Geometry: final body of the model. Coordinates: model frame, mm. Face numbers are marked on the shaded views. A direction names the side the tool comes from. Coordinates: 2 decimals unless noted, no trailing zeros. Loops run counter-clockwise (first coordinate to the right, second up) from the corner with the lowest first, then second, coordinate; pieces in that order, holes last. Notation, with made-up numbers: (77, 63) -> (100, 63) arc R11 cw to (100, 71) -> close; hole circle Ø11 at (-26, 2). An arc over 180 degrees is marked (long way). One line per item, written item: value. Start each with the question number.
Item 1: Contact query for flat-ended pins moving along their axis: pin 1 Ø2.5 at (x, y) = (-9, 34) entering from -Z; pin 2 Ø1.3 at (x, y) = (10.5, 7) entering from -Z. Output: stop coordinate, or through.
Item 2: Section query A-A on x = 0. Return loops of the section in (y, z), then the cut area to 3 significant figures.
Item 3: Set-up query: the marked faces 1, 2 and 3. Return all of +Z, -Z, +X, -X, +Y, -Y with unobstructed straight access to the full face (end or side cutting, diameter ignored); none if empty.
Item 4: Mould query, pull axis X, two halves, no side actions, for the marked faces 4, 5, 6 and 7. Classes: +X half, -X half, draft (parallel to the pull), parting line (faces both ways), or undercut.
Item 5: Ray query, probe 1 along Y at (x, z) = (0, 6.4); probe 2 along X at (y, z) = (21, 6.5); probe 3 along Y at (x, z) = (4.75, 4.75). Return the intervals inside material, ascending. Write a range as from..to.
Item 6: Section query B-B on y = 25.5. Return loops of the section in (x, z).
Item 7: Section query C-C on z = 3. Give the number of separate pieces and of enclosed holes in the cut face, then the cut area to 3 significant figures.
from build123d import *

# Parameters (mm, degrees)
EXTRUDE_1_DEPTH      = 7
EXTRUDE_1_DEPTH_BACK = 7
SKETCH_2_R           = 1.55
SKETCH_2_R_2         = 1.3
SKETCH_2_W           = 15.316718428
SKETCH_2_H           = 46.633436854
CUT_EXTRUDE_1_DEPTH  = 60.640590205
SKETCH_4_W           = 3.5
SKETCH_4_H           = 46.633436854
CUT_EXTRUDE_2_DEPTH  = 45.654227139
FILLET_1_R           = 2


with BuildPart() as part:
    # 草图2 → 凸台-拉伸1 (new, two sides: drawn at the far end of the back side and taken through both)
    with BuildSketch(Plane.XY.offset(-EXTRUDE_1_DEPTH_BACK)):
        with BuildLine():
            Line((9, 37), (-9, 37))
            ThreePointArc((-9, 37), (-11.121320344, 36.121320344), (-12, 34))
            Line((-12, 34), (-12, -18))
            ThreePointArc((-12, -18), (-11.121320344, -20.121320344), (-9, -21))
            Line((-9, -21), (9, -21))
            ThreePointArc((9, -21), (11.121320344, -20.121320344), (12, -18))
            Line((12, -18), (12, 34))
            ThreePointArc((12, 34), (11.121320344, 36.121320344), (9, 37))
        make_face()
        with Locations((-9, -18)):
            Circle(SKETCH_2_R, mode=Mode.SUBTRACT)
        with Locations((0, -18)):
            Circle(SKETCH_2_R_2, mode=Mode.SUBTRACT)
        with Locations((9, -18)):
            Circle(SKETCH_2_R, mode=Mode.SUBTRACT)
        with Locations((0, 8)):
            Rectangle(SKETCH_2_W, SKETCH_2_H, mode=Mode.SUBTRACT)
        with Locations((9, 34)):
            Circle(SKETCH_2_R, mode=Mode.SUBTRACT)
        with Locations((-9, 34)):
            Circle(SKETCH_2_R, mode=Mode.SUBTRACT)
    extrude(amount=EXTRUDE_1_DEPTH + EXTRUDE_1_DEPTH_BACK)

    # 草图3 → 切除-拉伸1 (cut, through all)
    with BuildSketch(Plane.XZ.offset(21)):
        with BuildLine():
            Line((-12, 0.5), (-5.979130372, 0.5))
            ThreePointArc((-5.979130372, 0.5), (0, 6), (5.979130372, 0.5))
            Line((5.979130372, 0.5), (12, 0.5))
            Line((12, 0.5), (12, -7))
            Line((12, -7), (-12, -7))
            Line((-12, -7), (-12, 0.5))
        make_face()
    extrude(amount=-CUT_EXTRUDE_1_DEPTH, mode=Mode.SUBTRACT)

    # 草图4 → 切除-拉伸2 (cut, through all)
    with BuildSketch(Plane.ZY.offset(12)):
        with Locations((2.25, 8)):
            Rectangle(SKETCH_4_W, SKETCH_4_H)
    extrude(amount=-CUT_EXTRUDE_2_DEPTH, mode=Mode.SUBTRACT)

    # 圆角1
    fillet_1_edges = [part.edges().sort_by_distance(p)[0] for p in [
        (7.658359214, 31.316718427, 5.5),
        (-7.658359214, 31.316718427, 5.5),
        (7.658359214, -15.316718427, 5.5),
        (-7.658359214, -15.316718427, 5.5),
        (-9.829179607, 31.316718427, 4),
        (-9.829179607, -15.316718427, 4),
        (9.829179607, -15.316718427, 4),
        (9.829179607, 31.316718427, 4),
    ]]
    fillet(fillet_1_edges, radius=FILLET_1_R)


solid = part.part
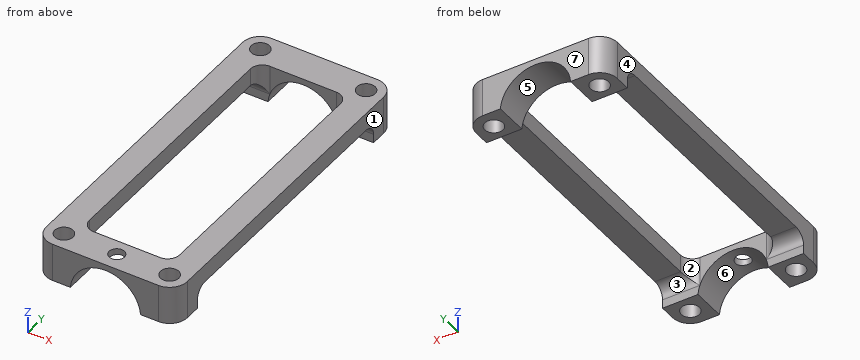
Reply:
1. pin 1: passes through
1. pin 2: stops at z = 4
2. outline: (-21, 6) -> (-19.3, 6) -> (-19.3, 7) -> (-21, 7) -> close; (-16.7, 6) -> (-15.32, 6) -> (-15.32, 7) -> (-16.7, 7) -> close; (31.32, 6) -> (37, 6) -> (37, 7) -> (31.32, 7) -> close
2. area: 8.77 mm²
3. face 1: +Z, -Z, +X, +Y, -Y
3. face 2: +Z, -Z
3. face 3: -Z, +X, -X
4. face 4: -X half
4. face 5: undercut
4. face 6: undercut
4. face 7: draft
5. probe 1: y = -21..-19.3, -16.7..-15.32, 31.32..37
5. probe 2: x = -12..-7.66, 7.66..12
5. probe 3: y = -21..-15.32, 31.32..37
6. outline: (-12, 4) -> (-7.66, 4) -> (-7.66, 7) -> (-12, 7) -> close; (7.66, 4) -> (12, 4) -> (12, 7) -> (7.66, 7) -> close
7. separate pieces: 4
7. enclosed holes: 4
7. area: 123 mm²
